Source: CAD feature listing. Evaluate the final solid. Frame: model axes, mm. Face numbers are marked on the shaded views. A direction names the side the tool comes from. Give positions to 0.01 mm unless a question says otherwise; leave off trailing zeros. Order: outer loops, then holes, each group sorted by start corner. A loop starts at its lowest first (then second) coordinate and runs counter-clockwise, first axis right, second up. Notation, with made-up numbers: (65, -11) -> (116, -11) arc R26 cw to (116, 15) -> close; hole circle Ø1 at (61, 13.25). An arc over 180 degrees is marked (long way). Use CSV: the item, a comma, the result in double quotes.
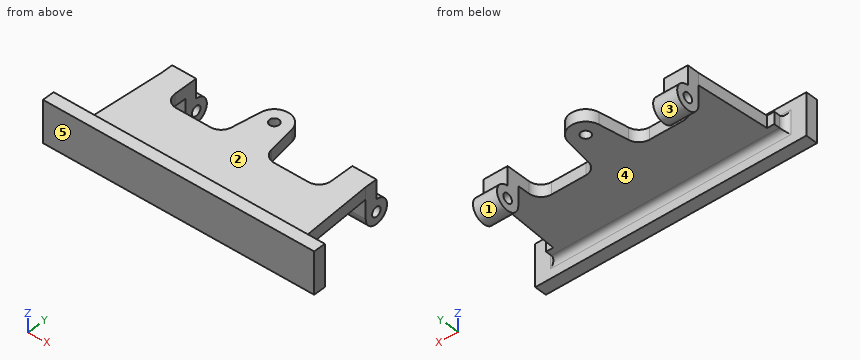
```python
from build123d import *

# Parameters (mm, degrees)
SKETCH1_R           = 4
BOSS_EXTRUDE1_DEPTH = 10
SKETCH2_W           = 225.743396996
SKETCH2_H           = 34.886278096
BOSS_EXTRUDE2_DEPTH = 10
SKETCH3_R           = 4
BOSS_EXTRUDE3_DEPTH = 20
FILLET1_R           = 5


with BuildPart() as part:
    # Sketch1 → Boss-Extrude1 (new body)
    with BuildSketch(Plane.XY):
        with BuildLine():
            Line((-85, -10), (-89, -70))
            Line((-89, -70), (-95, -70))
            Line((-95, -70), (-95, -80))
            Line((-95, -80), (95, -80))
            Line((95, -80), (95, -70))
            Line((95, -70), (89, -70))
            Line((89, -70), (85, -10))
            Line((85, -10), (65, -10))
            Line((65, -10), (65, -20))
            ThreePointArc((65, -20), (62.071067812, -27.071067812), (55, -30))
            Line((55, -30), (26.518096199, -30))
            ThreePointArc((26.518096199, -30), (20.033617948, -27.612591006), (16.645360037, -21.590308363))
            Line((16.645360037, -21.590308363), (12.83455701, 2.067400872))
            ThreePointArc((12.83455701, 2.067400872), (0, 13), (-12.83455701, 2.067400872))
            Line((-12.83455701, 2.067400872), (-16.645360037, -21.590308363))
            ThreePointArc((-16.645360037, -21.590308363), (-20.033617948, -27.612591006), (-26.518096199, -30))
            Line((-26.518096199, -30), (-55, -30))
            ThreePointArc((-55, -30), (-62.071067812, -27.071067812), (-65, -20))
            Line((-65, -20), (-65, -10))
            Line((-65, -10), (-85, -10))
        make_face()
        Circle(SKETCH1_R, mode=Mode.SUBTRACT)
    extrude(amount=BOSS_EXTRUDE1_DEPTH)

    # Sketch2 → Boss-Extrude2 (add)
    with BuildSketch(Plane(origin=(0, -80, 0), x_dir=(-1, 0, 0), z_dir=(0, -1, 0))):
        with Locations((0, -4.638757859)):
            Rectangle(SKETCH2_W, SKETCH2_H)
    extrude(amount=BOSS_EXTRUDE2_DEPTH)

    # Sketch3 → Boss-Extrude3 (add)
    with BuildSketch(Plane(origin=(-65, 0, 0), x_dir=(0, 0, -1), z_dir=(1, 0, 0))):
        with BuildLine():
            Line((6, 0), (-10, 0))
            Line((-10, 0), (-10, -10))
            Line((-10, -10), (16, -10))
            ThreePointArc((16, -10), (23.071067812, 7.071067812), (6, 0))
        make_face()
        with Locations(Location((16, 0, 0), (0, 0, 90))):
            Circle(SKETCH3_R, mode=Mode.SUBTRACT)
    boss_extrude3 = extrude(amount=-BOSS_EXTRUDE3_DEPTH)

    # Mirror1: Boss-Extrude3 across plane
    add(boss_extrude3.mirror(Plane(origin=(0, 0, 0), x_dir=(0, 0, 1), z_dir=(1, 0, 0))))

    # Fillet1
    fillet1_edges = [part.edges().sort_by_distance(p)[0] for p in [
        (0, -80, 0),
        (95, -80, 5),
        (-95, -80, 5),
        (0, -80, 10),
    ]]
    fillet(fillet1_edges, radius=FILLET1_R)


solid = part.part
```
1. Mould query, pull axis Y, two halves, no side actions, for the marked faces 3, 4 and 5. Classes: released by +Y, released by -Y, zero draft, split by the parting line, or undercut.
Answer below:
face 3,"split by the parting line"
face 4,"undercut"
face 5,"released by -Y"
2. Section query D-D on y = -65. Return loops of the section in (x, z), plus the area to 3 significant figures.
Answer below:
outline,"(-88.67, 0) -> (88.67, 0) -> (88.67, 10) -> (-88.67, 10) -> close"
area,"1,770 mm²"
3. Ray query, line 1 along Y through (x, z) = (0, 3.75); line 2 along X through (y, z) = (-7, -13.5); line 3 along Z through (x, y) = (35.5, -39.5). Return the intervals inside material, ascending.
Answer below:
line 1,"y = -90 to -4, 4 to 13"
line 2,"x = -85 to -65, 65 to 85"
line 3,"z = 0 to 10"
4. Section query C-C on y = -51. Return loops of the section in (x, z), plus the area to 3 significant figures.
Answer below:
outline,"(-87.73, 0) -> (87.73, 0) -> (87.73, 10) -> (-87.73, 10) -> close"
area,"1,750 mm²"
5. Section query A-A on x = 0. Return loops of the section in (y, z).
Answer below:
outline,"(-90, -12.8) -> (-80, -12.8) -> (-80, -5) arc R5 cw to (-75, 0) -> (-4, 0) -> (-4, 10) -> (-75, 10) arc R5 cw to (-80, 15) -> (-80, 22.08) -> (-90, 22.08) -> close; (4, 0) -> (13, 0) -> (13, 10) -> (4, 10) -> close"
6. Pin query (flat end, axial travel): P1, Ø11, axis at x = 43, z = 5, coming from the +Y side; P2, Ø4, axis at y = -73.5, z = 5.5, coming from the +X side; P3, Ø6, axis at y = -41, z = 9.5, coming from the +X side; P4, Ø7, axis at y = 0, z = -16, coming from the +X side. Return the tip coordinate at first contact, or that it passes through.
Answer below:
P1,"stops at y = -30"
P2,"stops at x = 95.03"
P3,"stops at x = 87.27"
P4,"passes through"
7. Section query B-B on x = 48. Return loops of the section in (y, z), plus the area to 3 significant figures.
Answer below:
outline,"(-90, -12.8) -> (-80, -12.8) -> (-80, -5) arc R5 cw to (-75, 0) -> (-30, 0) -> (-30, 10) -> (-75, 10) arc R5 cw to (-80, 15) -> (-80, 22.08) -> (-90, 22.08) -> close"
area,"860 mm²"
8. Access query for the marked faces 1 and 2. Directions: +Z, -Z, +X, -X, +Y, -Y. A direction counts if a zero-diameter tool reaches every point of the face in a straight line with its end or side. Return the directions, or none.
Answer below:
face 1,"+X, -X"
face 2,"+Z, +X, -X, +Y"
